Could you check a few things on this model? Use its own coordinates, in mm. A direction names the side the tool comes from. Round coordinates to 2 decimals unless told otherwise and drop trailing zeros. Loops run counter-clockwise (first coordinate to the right, second up) from the corner with the lowest first, then second, coordinate; pieces in that order, holes last.
from build123d import *

# Parameters (mm, degrees)
SKETCH1_W               = 25
SKETCH1_H               = 7
CUT_EXTRUDE1_DEPTH      = 213.265164358
CUT_EXTRUDE1_DEPTH_BACK = 213.265164358
SKETCH2_R               = 1.5
CHAMFER1_SIZE           = 1


with BuildPart() as part:
    # Sketch1 → Revolve1 (revolve)
    with BuildSketch(Plane(origin=(0, 0, 0), x_dir=(0, 0, -1), z_dir=(1, 0, 0)), mode=Mode.PRIVATE) as revolve1_sk:
        with Locations((12.5, 3.5)):
            Rectangle(SKETCH1_W, SKETCH1_H)
        Polygon((25, 7), (25, 0), (187, 0), (187, 7), (187, 7.5), (25, 7.5), align=None)
        with Locations((199.5, 3.5)):
            Rectangle(SKETCH1_W, SKETCH1_H)
    revolve(revolve1_sk.sketch.rotate(Axis((0, 0, -25), (0, 0, -1)), 90), axis=Axis((0, 0, -25), (0, 0, -1)))

    # Sketch2 → Cut-Extrude1 (cut, two sides: drawn at the far end of the back side and taken through both)
    with BuildSketch(Plane(origin=(0, 0, 0), x_dir=(0, 0, -1), z_dir=(1, 0, 0)).offset(-CUT_EXTRUDE1_DEPTH_BACK)):
        with Locations((5, 0)):
            Circle(SKETCH2_R)
        with Locations((207, 0)):
            Circle(SKETCH2_R)
    extrude(amount=CUT_EXTRUDE1_DEPTH + CUT_EXTRUDE1_DEPTH_BACK, mode=Mode.SUBTRACT)

    # Chamfer1
    chamfer1_edges = [part.edges().sort_by_distance(p)[0] for p in [
        (-7, 0, 0),
        (-7, 0, -212),
    ]]
    chamfer(chamfer1_edges, length=CHAMFER1_SIZE)


solid = part.part
Item 1: If I drill on line 1 along Z through (x, y) = (-2.75, 0); line 2 along Z through (x, y) = (-4, -1.25); line 3 along Y through (x, z) = (-0.25, -207), over which ranges is the centre line in solid material (lowest first)?
Results list:
line 1: z = -212 to -208.5, -205.5 to -6.5, -3.5 to 0
line 2: z = -212 to -207.83, -206.17 to -5.83, -4.17 to 0
line 3: y = -7 to -1.5, 1.5 to 7
Item 2: If we section it at C-C, the plane z = -59.5: Please give me the cut outline in (x, y).
Results list:
outline: circle Ø15 at (0, 0)
Item 3: If we section it at A-A, the plane x = 0: Please give me the cut outline in (y, z), then the cut area to 3 significant figures.
Results list:
outline: (-7.5, -187) - (-7, -187) - (-7, -211) - (-6, -212) - (6, -212) - (7, -211) - (7, -187) - (7.5, -187) - (7.5, -25) - (7, -25) - (7, -1) - (6, 0) - (-6, 0) - (-7, -1) - (-7, -25) - (-7.5, -25) - close; hole circle Ø3 at (0, -207); hole circle Ø3 at (0, -5)
area: 3,110 mm2
Item 4: If we section it at B-B, the plane z = -15.5: Please give me the cut outline in (x, y).
Results list:
outline: circle Ø14 at (0, 0)
Item 5: Will these pins go through, and if not, where does the flat tip stop? pin 1 (8 mm diameter, centred on x = 5, y = -5, fed in from +Z); pin 2 (3 mm diameter, centred on x = -3.5, z = -132, fed in from -Y); pin 3 (1 mm diameter, centred on y = 5.5, z = -47.5, fed in from +X).
Results list:
pin 1: stops at z = 0
pin 2: stops at y = -7.23
pin 3: stops at x = 5.59
Item 6: For faces 1 (the flat face through (2, 7, -187)), 2 (the flat face through (0, 0, -212)), 3 (the cylindrical face through (6.677, -2.103, -13.168)), which set-ups out of +Z, -Z, +X, -X, +Y, -Y let a thin tool reach every point of the face, with its end or its side?
Results list:
face 1: -Z
face 2: -Z, +X, -X, +Y, -Y
face 3: +Z
